Source: CAD feature listing. Evaluate the final solid. Frame: model axes, mm. A direction names the side the tool comes from. Round coordinates to 2 decimals unless told otherwise and drop trailing zeros. Order: outer loops, then holes, each group sorted by start corner. A loop starts at its lowest first (then second) coordinate and runs counter-clockwise, first axis right, second up. Notation, with made-up numbers: M -19,62 L 26,62 A32 ccw 26,96 Z; hole C 42,62.25 d1. An arc over 180 degrees is marked long. Use CSV: the item, a comma, the result in double quotes. Start each with the question number.
```python
from build123d import *

# Parameters (mm, degrees)
SKETCH1_W                                            = 12
SKETCH1_H                                            = 7.5
BOSS_EXTRUDE1_DEPTH                                  = 185
CHAMFER1_SIZE                                        = 0.5
HOLE_SIZE_PER_SOCKET_HEAD_CAP_SCREW_TYPE_D           = 3.4
HOLE_SIZE_PER_SOCKET_HEAD_CAP_SCREW_TYPE_CBORE_D     = 6
HOLE_SIZE_PER_SOCKET_HEAD_CAP_SCREW_TYPE_CBORE_DEPTH = 3.4
LPATTERN1_COUNT                                      = 8
LPATTERN1_PITCH                                      = 25


with BuildPart() as part:
    # Sketch1 → Boss-Extrude1 (new body)
    with BuildSketch(Plane.XY):
        Rectangle(SKETCH1_W, SKETCH1_H)
    extrude(amount=BOSS_EXTRUDE1_DEPTH)

    # Chamfer1
    chamfer1_edges = [part.edges().sort_by_distance(p)[0] for p in [
        (6, -3.75, 92.5),
        (-6, -3.75, 92.5),
    ]]
    chamfer(chamfer1_edges, length=CHAMFER1_SIZE)

    # Hole size per socket head cap screw type1 (through all)
    with Locations(Plane(origin=(0, 3.75, 0), x_dir=(-1, 0, 0), z_dir=(0, 1, 0))):
        with Locations((0, 5)):
            hole_size_per_socket_head_cap_screw_type = CounterBoreHole(HOLE_SIZE_PER_SOCKET_HEAD_CAP_SCREW_TYPE_D / 2, HOLE_SIZE_PER_SOCKET_HEAD_CAP_SCREW_TYPE_CBORE_D / 2, HOLE_SIZE_PER_SOCKET_HEAD_CAP_SCREW_TYPE_CBORE_DEPTH)

    # LPattern1: Hole size per socket head cap screw type1 ×8
    with Locations(*[(0, 0, i * LPATTERN1_PITCH) for i in range(1, LPATTERN1_COUNT)]):
        add(hole_size_per_socket_head_cap_screw_type, mode=Mode.SUBTRACT)


solid = part.part
```
(1) Section A-A on z = 180. Return loops of the section in (x, y).
(2) Line query: line 1 along X through (y, z) = (1.25, 156.5); line 2 along Y through (x, z) = (-2.25, 154); line 3 along X through (y, z) = (1, 82.5). Output: solid intervals per line, ascending.
(3) Section B-B on y = -1.25. Give the number of separate pieces and of enclosed holes in the cut face, plus the area to 3 significant figures.
(4) Draft query along Z for faces 1 (the face through (0, 0.35, 28)), 2 (the face through (0, 0, 0)), 3 (the face through (6, 0, 91)). Return one class per face: pulls with the +Z half, pulls with the -Z half, needs draft (parallel to the pull), parting line crosses it, or undercut.
(5) Reachability of faces 4 (the face through (0, 0.35, 53)), 5 (the face through (-0.37, -1.73, 178.34)) from +Z, -Z, +X, -X, +Y, -Y: full face, straight path, thin tool, end or side. Return the list, or none.
(6) Contact query for a flat-ended pin moving along its axis: P1, Ø3, axis at x = 0.5, z = 4, coming from the +Y side. Output: stop coordinate, or through.
Results below:
1,outline,"M -6,-3.25 L -5.5,-3.75 L -1.7,-3.75 L -1.7,0.35 L -3,0.35 L -3,3.75 L -6,3.75 Z; M 1.7,-3.75 L 5.5,-3.75 L 6,-3.25 L 6,3.75 L 3,3.75 L 3,0.35 L 1.7,0.35 Z"
2,line 1,"x = -6 to -2.6, 2.6 to 6"
2,line 2,"y = -3.75 to 0.35"
2,line 3,"x = -6 to -1.66, 1.66 to 6"
3,separate pieces,"1"
3,enclosed holes,"8"
3,area,"2,150 mm2"
4,face 1,"undercut"
4,face 2,"pulls with the -Z half"
4,face 3,"needs draft"
5,face 4,"+Y"
5,face 5,"+Y, -Y"
6,P1,"stops at y = 0.35"
